```python
from build123d import *

# Parameters (mm, degrees)
SKETCH5_W           = 13.145964729
SKETCH5_H           = 100
SKETCH6_R           = 28
BOSS_EXTRUDE1_DEPTH = 10
SKETCH7_R           = 2
CUT_EXTRUDE1_DEPTH  = 10
CIRPATTERN1_COUNT   = 10


with BuildPart() as part:
    # Sketch4 → Revolve1 (revolve)
    with BuildSketch(Plane(origin=(20, 0, 0), x_dir=(0, -1, 0), z_dir=(-1, 0, 0)), mode=Mode.PRIVATE) as revolve1_sk:
        Polygon((-76.830512452, 0), (-76.830512452, -4.383431838), (-68.830512452, -11.214554774), (-69.034523253, -121.214554774), (-55.830512452, -121.214554774), (-55.830512452, 15), (-78.802692797, 15), (-78.830512452, 0), align=None)
    revolve(revolve1_sk.sketch.rotate(Axis((20, 55.830512452, 15), (0, 0, -1)), 90), axis=Axis((20, 55.830512452, 15), (0, 0, -1)))

    # Sketch5 → Cut-Revolve1 (revolve, cut)
    with BuildSketch(Plane(origin=(20, 0, 0), x_dir=(0, -1, 0), z_dir=(-1, 0, 0)), mode=Mode.PRIVATE) as cut_revolve1_sk:
        with Locations((-42.728507052, -66.214554774)):
            Rectangle(SKETCH5_W, SKETCH5_H)
    revolve(cut_revolve1_sk.sketch.rotate(Axis((20, 55.830512452, -11.214554774), (0, 0, -1)), 270), axis=Axis((20, 55.830512452, -11.214554774), (0, 0, -1)), mode=Mode.SUBTRACT)

    # Sketch6 → Boss-Extrude1 (add)
    with BuildSketch(Plane(origin=(0, 0, 15), x_dir=(-1, 0, 0), z_dir=(0, 0, -1))):
        with Locations((-20, 55.830512452)):
            Circle(SKETCH6_R)
    extrude(amount=BOSS_EXTRUDE1_DEPTH)

    # Sketch7 → Cut-Extrude1 (cut)
    with BuildSketch(Plane(origin=(0, 0, 5), x_dir=(-1, 0, 0), z_dir=(0, 0, -1))):
        with Locations((4.75295766, 51.209902338)):
            Circle(SKETCH7_R)
    cut_extrude1 = extrude(amount=-CUT_EXTRUDE1_DEPTH, mode=Mode.SUBTRACT)

    # CirPattern1: Cut-Extrude1 ×10 about axis
    cirpattern1_axis = Axis((20, 55.830512452, 0), (0, 0, 1))
    for i in range(1, CIRPATTERN1_COUNT):
        add(cut_extrude1.rotate(cirpattern1_axis, i * 360 / CIRPATTERN1_COUNT), mode=Mode.SUBTRACT)


solid = part.part
```
Input: part model. Units: mm. Frame: model coordinates. A direction names the side the tool comes from. Round coordinates to 2 decimals unless told otherwise and drop trailing zeros. Order: outer loops, then holes, each group sorted by start corner. A loop starts at its lowest first (then second) coordinate and runs counter-clockwise, first axis right, second up. Notation, with made-up numbers: (-13.5, -8.75) - (-5.5, -8.75) arc R26 cw to (-5.5, 15.25) - close; hole circle Ø6 at (-2, 89). An arc over 180 degrees is marked (long way). Answer in a Markdown table with one row per item.
Item 1: Section query A-A (z = -82). Return the cut outline in (x, y).
Model answer:
| item | result |
|---|---|
| outline | circle Ø13.06 at (20, 55.83) |
Item 2: Pin query (flat end, axial travel): pin 1 (6 mm diameter, centred on x = 15, z = -100.5, fed in from -Y); pin 2 (12 mm diameter, centred on x = 12.5, z = -63, fed in from -Y); pin 3 (1.5 mm diameter, centred on x = 20.5, z = -67, fed in from -Y). Return the tip coordinate at first contact, or that it passes through.
Model answer:
| item | result |
|---|---|
| pin 1 | stops at y = 49.62 |
| pin 2 | stops at y = 49.48 |
| pin 3 | stops at y = 49.3 |
Item 3: Reachability of faces 1 (the conical face through (32.013, 60.811, -13.75)), 2 (the cylindrical face through (44.49, 58.47, 9.93)), 3 (the cylindrical face through (3.335, 68.609, -2.222)) from +Z, -Z, +X, -X, +Y, -Y: full face, straight path, thin tool, end or side. Return the list, or none.
Model answer:
| item | result |
|---|---|
| face 1 | none |
| face 2 | +Z, -Z |
| face 3 | -Z |
Item 4: Mould query, pull axis Z, two halves, no side actions, for faces 4 (the cylindrical face through (1.735, 39.3, 9.93)), 5 (the flat face through (20, 56, 15)), 6 (the flat face through (20, 56, -121.215)), 7 (the conical face through (26.09, 67.54, -118.75)). Classes: released by +Z, released by -Z, zero draft, split by the parting line, or undercut.
Model answer:
| item | result |
|---|---|
| face 4 | zero draft |
| face 5 | released by +Z |
| face 6 | released by -Z |
| face 7 | undercut |
Item 5: Line query: line 1 (Z direction, x = 11, y = 54.5); line 2 (Y direction, x = 20.5, z = 9); line 3 (Y direction, x = 20, z = -81). Output: solid intervals per line, ascending.
Model answer:
| item | result |
|---|---|
| line 1 | z = -121.21 to -116.21, -16.21 to 15 |
| line 2 | y = 27.83 to 83.83 |
| line 3 | y = 49.3 to 62.36 |
